Design review of the part built by this model. Coordinates are the model's own, in mm. A direction names the side the tool comes from. Coordinates: 2 decimals unless noted, no trailing zeros. Write each loop counter-clockwise with the first axis right and the second up, starting at its lowest first coordinate (ties: lowest second). Pieces come first, ordered by that corner, then holes. Notation, with made-up numbers: (57, -19) - (82, -19) arc R11 ccw to (82, -9) - close; hole circle Ø6 at (28.25, 67.25). An arc over 180 degrees is marked (long way). Answer as CSV lines item,"result". Start each with the question number.
Q1. For line 1 along Y through (x, z) = (-4, 2); line 2 along Y through (x, z) = (-14, -4.5); line 3 along X through (y, z) = (30, -4.5), list the stretches that pass through material, from the lowest coordinate up. Write a range as [from, to].
Q2. We need section B-B (z = 8). Write out the cut boundary in (x, y), plus the area to 3 significant figures.
Q3. Clearance check with flat-ended pins moving along their axes: pin 1 (1.5 mm diameter, centred on y = -2, z = 13.5, fed in from -X); pin 2 (2.5 mm diameter, centred on x = -17, z = -4.5, fed in from -Y); pin 3 (10 mm diameter, centred on x = -9.5, y = 15.5, fed in from -Z); pin 4 (5 mm diameter, centred on x = 2.5, z = 0.5, fed in from +Y). State where each tip first meets the part, or that it passes through.
Q4. We need section C-C (x = -3). Write out the cut boundary in (y, z).
Q5. We need section D-D (y = 13.5). Write out the cut boundary in (x, z).
Q6. Mouldability with a two-part tool opening along X and no side actions: class faces 4 (the face through (16, 38, 0)), 5 (the face through (0, 22, 0)), 6 (the face through (-20, 15, 0)) as pulls with the +X half, pulls with the -X half, needs draft (parallel to the pull), parting line crosses it, or undercut.
Q7. Machinability: for faces 1 (the face through (0, 15, 15)), 2 (the face through (-16, 0, 0)), 3 (the face through (16, 0, 0)), which of the approach directions +Z, -Z, +X, -X, +Y, -Y give a long, thin tool a straight path to every point of the face, cutting with its end or side? Answer none if there is none.
Q8. We need section A-A (y = 30). Write out the cut boundary in (x, z), plus the area to 3 significant figures.
from build123d import *

# Parameters (mm, degrees)
BASE_BLOCK_30MM_DEPTH  = 15
GROOVE_CUT_40MM_DEPTH  = 20
FRONT_BLOCK_SKETCH_W   = 24
FRONT_BLOCK_SKETCH_H   = 23
FRONT_BLOCK_38MM_DEPTH = 19


with BuildPart() as part:
    # Base Profile Sketch → Base Block 30mm (new, symmetric)
    with BuildSketch(Plane.XY):
        Polygon((8, 22), (12, 38), (20, 38), (20, 0), (0, 0), (-20, 0), (-20, 38), (-12, 38), (-8, 22), align=None)
    extrude(amount=BASE_BLOCK_30MM_DEPTH, both=True)

    # Groove Profile Sketch → Groove Cut 40mm (cut, symmetric)
    with BuildSketch(Plane(origin=(0, 0, 0), x_dir=(0, 0, -1), z_dir=(1, 0, 0))):
        Polygon((-15, 0), (-7, 38), (-15, 38), align=None)
        Polygon((15, 38), (15, 0), (7, 38), align=None)
    extrude(amount=GROOVE_CUT_40MM_DEPTH, both=True, mode=Mode.SUBTRACT)

    # Front Block Sketch → Front Block 38mm (add, symmetric)
    with BuildSketch(Plane.XY):
        with Locations((0, 3.5)):
            Rectangle(FRONT_BLOCK_SKETCH_W, FRONT_BLOCK_SKETCH_H)
    extrude(amount=FRONT_BLOCK_38MM_DEPTH, both=True)


solid = part.part
Results list:
1,line 1,"y = [-8, 22]"
1,line 2,"y = [0, 38]"
1,line 3,"x = [-20, -10], [10, 20]"
2,outline,"(-20, 0) - (-12, 0) - (-12, -8) - (12, -8) - (12, 0) - (20, 0) - (20, 33.25) - (10.81, 33.25) - (8, 22) - (-8, 22) - (-10.81, 33.25) - (-20, 33.25) - close"
2,area,"1,310 mm2"
3,pin 1,"stops at x = -12"
3,pin 2,"stops at y = 0"
3,pin 3,"stops at z = -19"
3,pin 4,"stops at y = 22"
4,outline,"(-8, -19) - (15, -19) - (15, -11.84) - (22, -10.37) - (22, 10.37) - (15, 11.84) - (15, 19) - (-8, 19) - close"
5,outline,"(-20, -12.16) - (-12, -12.16) - (-12, -19) - (12, -19) - (12, -12.16) - (20, -12.16) - (20, 12.16) - (12, 12.16) - (12, 19) - (-12, 19) - (-12, 12.16) - (-20, 12.16) - close"
6,face 4,"needs draft"
6,face 5,"undercut"
6,face 6,"pulls with the -X half"
7,face 1,"+Z, +X, -X, +Y"
7,face 2,"+Z, -Z, -X, -Y"
7,face 3,"+Z, -Z, +X, -Y"
8,outline,"(-20, -8.68) - (-10, -8.68) - (-10, 8.68) - (-20, 8.68) - close; (10, -8.68) - (20, -8.68) - (20, 8.68) - (10, 8.68) - close"
8,area,"347 mm2"
